Could you check a few things on this drawing? It's one solid part, dimensions in mm from its lowest x, y, z. A direction names the side the tool comes from. Coordinates: 2 decimals unless noted, no trailing zeros. Order: outer loops, then holes, each group sorted by start corner. A loop starts at its lowest first (then second) coordinate and runs counter-clockwise, first axis right, second up. Notation, with made-up numbers: M -35.5,4 L 1.5,4 A26 ccw 1.5,36 Z; hole C -10,8 d6. An arc over 180 degrees is marked long. Answer as CSV lines item,"result". Start each with the question number.
1. If we section it at A-A (z = 20): List the corners of the cut face in (x, y) for me, plus the area to 3 significant figures.
2. On a 3-axis mill with a long thin cutter (end or side, diameter ignored), from which of +Z, -Z, +X, -X, +Y, -Y can I reach the whole of each face in a straight line? I mean the marked faces 1 and 2. Say none if no direction works.
3. If we section it at D-D (z = 30.5): List the corners of the cut face in (x, y) for me, plus the area to 3 significant figures.
4. I need wall thicknesses on line 1 along X through (y, z) = (13.25, 20); line 2 along Y through (x, z) = (96, 7.5); line 3 along Z through (x, y) = (65, 14.25). Which ranges of each line are inside material? Lowest first, please. Write a range as from..to.
5. Will these pins go through, and if not, where does the flat tip stop? pin 1 (11 mm diameter, centred on x = 65, z = 20, fed in from +Y); pin 2 (6 mm diameter, centred on x = 31, z = 9, fed in from -Y).
6. If we section it at B-B (x = 65): List the corners of the cut face in (y, z) for me.
7. If we section it at C-C (y = 11.75): List the corners of the cut face in (x, z) for me.
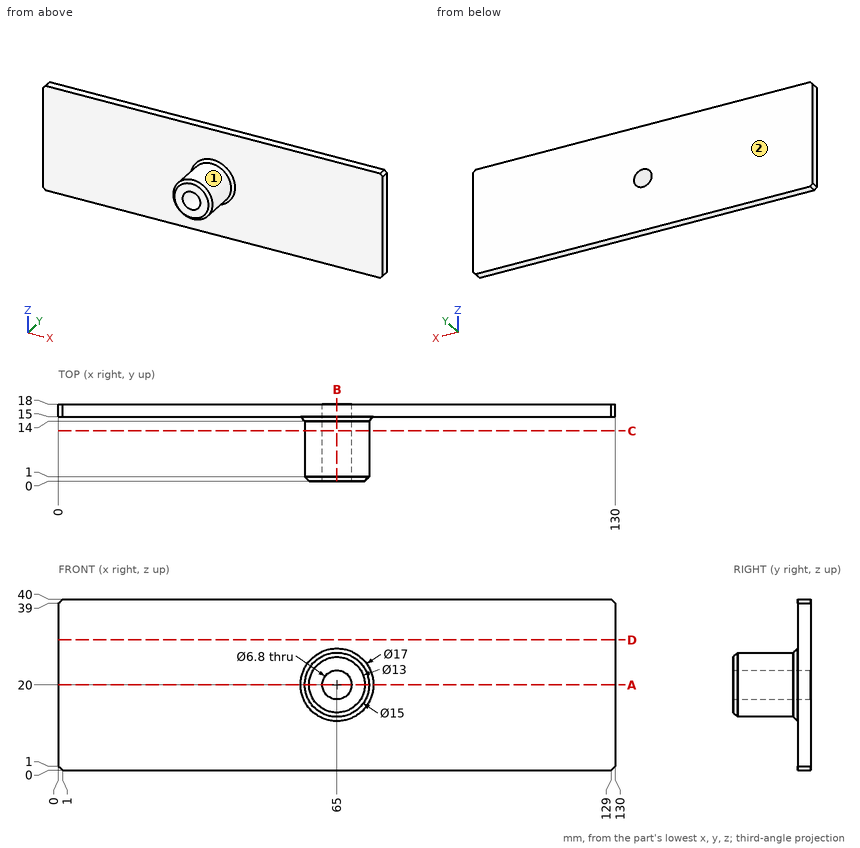
Solved:
1,outline,"M 0,15 L 56.5,15 L 57.5,14 L 57.5,1 L 58.5,0 L 61.6,0 L 61.6,18 L 0,18 Z; M 68.4,0 L 71.5,0 L 72.5,1 L 72.5,14 L 73.5,15 L 130,15 L 130,18 L 68.4,18 Z"
1,area,"493 mm²"
2,face 1,"-Y"
2,face 2,"+Z, -Z, +X, -X, +Y"
3,outline,"M 0,15 L 130,15 L 130,18 L 0,18 Z"
3,area,"390 mm²"
4,line 1,"57.5..61.6, 68.4..72.5"
4,line 2,"15..18"
4,line 3,"12.25..16.6, 23.4..27.75"
5,pin 1,"y = 18"
5,pin 2,"y = 15"
6,outline,"M 0,13.5 L 1,12.5 L 14,12.5 L 15,11.5 L 15,0 L 18,0 L 18,16.6 L 0,16.6 Z; M 0,23.4 L 18,23.4 L 18,40 L 15,40 L 15,28.5 L 14,27.5 L 1,27.5 L 0,26.5 Z"
7,outline,"C 65,20 d15; hole C 65,20 d6.8"
